from build123d import *

# Parameters (mm, degrees)
SKETCH_1_W                   = 180
SKETCH_1_H                   = 730
EXTRUDE_1_DEPTH              = 10
HOLE_WIZARD_M5_1_D           = 5.5
HOLE_WIZARD_M5_1_CBORE_D     = 10
HOLE_WIZARD_M5_1_CBORE_DEPTH = 5.4
MM_0_D                       = 5
CHAMFER_1_SIZE               = 10
HOLE_WIZARD_M5_2_D           = 4.2
HOLE_WIZARD_M5_3_D           = 4.2
HOLE_WIZARD_M4_1_D           = 3.3
EXTRUDE_2_DEPTH              = 10


with BuildPart() as part:
    # 草图1 → 凸台-拉伸1 (new body)
    with BuildSketch(Plane.XY):
        Rectangle(SKETCH_1_W, SKETCH_1_H)
    extrude(amount=EXTRUDE_1_DEPTH)

    # M5 六角凹头螺钉的柱形沉头孔1 (through all)
    with Locations(Plane.XY.offset(10)):
        with Locations((-37, -200), (37, -200), (-37, -295), (37, -295)):
            CounterBoreHole(HOLE_WIZARD_M5_1_D / 2, HOLE_WIZARD_M5_1_CBORE_D / 2, HOLE_WIZARD_M5_1_CBORE_DEPTH)

    # 大小mm 暗销孔0 (through all)
    with Locations(Plane.XY.offset(10)):
        with Locations((0, -200), (0, -295)):
            Hole(MM_0_D / 2)

    # 倒角1
    chamfer_1_edges = [part.edges().sort_by_distance(p)[0] for p in [
        (90, -365, 5),
        (-90, -365, 5),
        (-90, 365, 5),
        (90, 365, 5),
    ]]
    chamfer(chamfer_1_edges, length=CHAMFER_1_SIZE)

    # M5 螺纹孔2 (through all)
    with Locations(Plane.XY.offset(10)):
        with Locations((80, 293), (-2, 293), (80, 93), (80, 43), (-2, 43), (-2, 93)):
            Hole(HOLE_WIZARD_M5_2_D / 2)

    # M5 螺纹孔3 (through all)
    with Locations(Plane(origin=(0, 0, 0), x_dir=(-1, 0, 0), z_dir=(0, 0, -1))):
        with Locations((-17.5, -105.532443279), (-17.5, -145.532443279), (17.5, -105.532443279), (17.5, -145.532443279)):
            Hole(HOLE_WIZARD_M5_3_D / 2)

    # M4 螺纹孔1 (through all)
    with Locations(Plane.XY.offset(10)):
        with Locations((-81.499026454, 34.792936996), (-59.499927509, 34.792936996), (-77.499026454, 34.792936996), (-63.499026454, 34.792936996)):
            Hole(HOLE_WIZARD_M4_1_D / 2)

    # 草图12 → 凸台-拉伸2 (add)
    with BuildSketch(Plane.ZY.offset(90)):
        Polygon((0, -65), (-50, -365), (0, -365), align=None)
    extrude_2 = extrude(amount=-EXTRUDE_2_DEPTH)

    # 镜向1: 凸台-拉伸2 across plane
    add(extrude_2.mirror(Plane(origin=(0, 0, 0), x_dir=(0, 0, 1), z_dir=(1, 0, 0))))


solid = part.part
CAD build for the part. Positions are in the model's coordinates, mm. A direction names the side the tool comes from. Round coordinates to 2 decimals unless told otherwise and drop trailing zeros. Write each loop counter-clockwise with the first axis right and the second up, starting at its lowest first coordinate (ties: lowest second). Pieces come first, ordered by that corner, then holes. Notation, with made-up numbers: (47, 25.5) -> (88, 25.5) arc R25 ccw to (88, 50.5) -> close; hole circle Ø11 at (63, 82.5). An arc over 180 degrees is marked (long way). Answer as a JSON object with one key per item and string values.
(1) Two-plate mould, pull along X, no slides. Class faces 1 (the face through (85.07, -212.9, -24.65)), 2 (the face through (90, -137, -2)), 3 (the face through (80, -280, -14)): +X half, -X half, draft (parallel to the pull), parting line (faces both ways), or undercut.
Reported:
{"face 1": "draft", "face 2": "+X half", "face 3": "undercut"}
(2) Probe probe 1 along X at (y, z) = (293, 5.25); probe 2 along Y at (x, z) = (37, 2.85); probe 3 along Y at (x, z) = (80, 3.75). List the from-to ranges inside material, lowest first. Write a range as [from, to].
Reported:
{"probe 1": "x = [-90, -4.1], [0.1, 77.9], [82.1, 90]", "probe 2": "y = [-365, -297.75], [-292.25, -202.75], [-197.25, 365]", "probe 3": "y = [-365, 40.9], [45.1, 90.9], [95.1, 290.9], [295.1, 365]"}
(3) Pin check, flat tips, straight feed: P1, Ø3, axis at x = 0, y = -295, coming from the -Z side; P2, Ø5, axis at x = 80, y = 293, coming from the +Z side; P3, Ø9, axis at x = 37, y = -200, coming from the -Z side; P4, Ø3, axis at x = -38, y = -293, coming from the +Z side. Stop position of each tip, or through.
Reported:
{"P1": "passes through", "P2": "stops at z = 10", "P3": "stops at z = 0", "P4": "stops at z = 4.6"}
(4) Which spindle directions (+Z, -Z, +X, -X, +Y, -Y) get a long thin tool onto all of the face, cutting with end or side? Do faces 4 (the face through (-80, -280, -14)), 5 (the face through (-90, -137, -2)). Say none if no direction does.
Reported:
{"face 4": "-Z, +Y, -Y", "face 5": "+Z, -Z, -X, +Y, -Y"}
(5) Band-saw the part on A-A, the plane z = -35. List the corners of the cut face in (x, y).
Reported:
{"outline": "(-90, -365) -> (-80, -365) -> (-80, -275) -> (-90, -275) -> close; (80, -365) -> (90, -365) -> (90, -275) -> (80, -275) -> close"}
(6) Band-saw the part on B-B, the plane y = 64.5. List the corners of the cut face in (x, z).
Reported:
{"outline": "(-90, 0) -> (90, 0) -> (90, 10) -> (-90, 10) -> close"}
